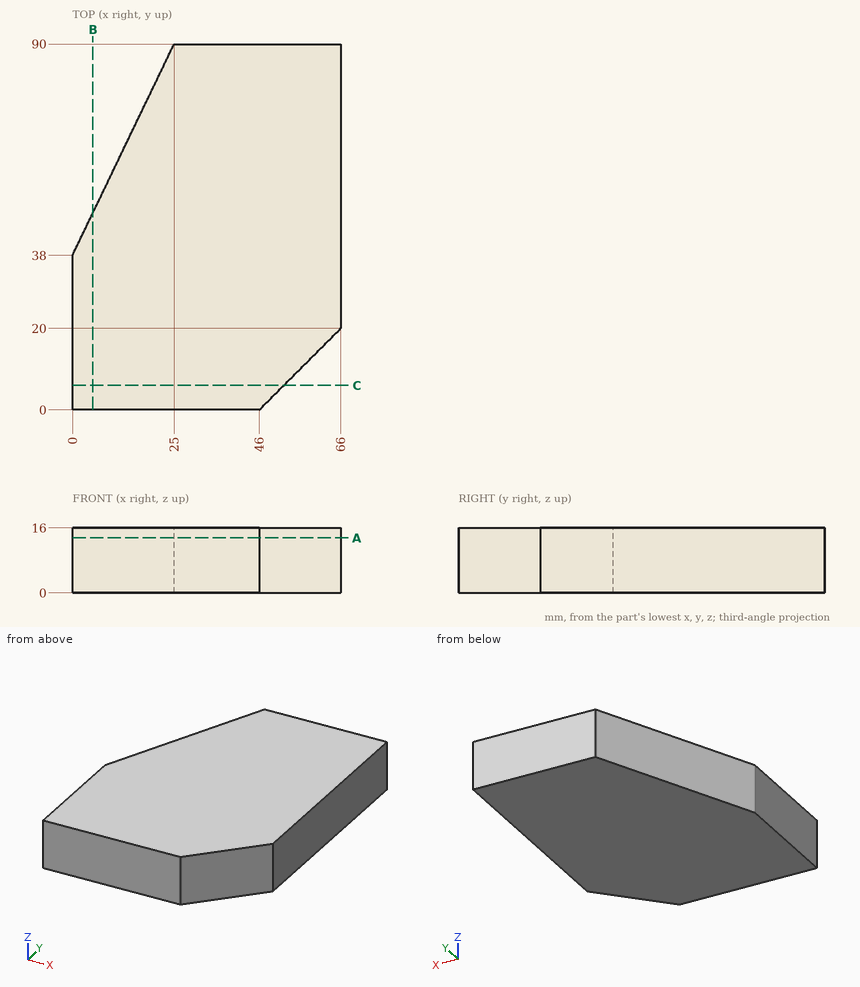
Input: dimensioned drawing with shaded views. Units: mm. Origin: part minimum x, y, z. Coordinates: 2 decimals unless noted, no trailing zeros. Loops run counter-clockwise (first coordinate to the right, second up) from the corner with the lowest first, then second, coordinate; pieces in that order, holes last. Notation, with made-up numbers: M 1.25,20.25 L 57.25,20.25 A5 cw 57.25,25.25 Z; hole C 70.5,10 d9. An arc over 180 degrees is marked long. Use a Markdown table: item, result. Add a question column.
Q1. Section query A-A, the plane z = 13.5. Return loops of the section in (x, y).
Q2. Section query C-C, the plane y = 6. Return loops of the section in (x, z), and give its area (3 significant figures).
Q3. Material intervals for L1, parallel to Y at x = 55.5, z = 1.5; L2, parallel to X at y = 7, z = 11.25; L3, parallel to Y at x = 9.5, z = 6.5, sorted ascending.
Q4. Section query B-B, the plane x = 5. Return loops of the section in (y, z).
Q5. First-contact query: pin 1 (2 mm diameter, centred on y = 50.5, z = 4.5, fed in from -X); pin 2 (5 mm diameter, centred on y = 67.5, z = 7.5, fed in from -X). Flat tips, straight axial feed; report the tip coordinate or a pass-through.
Result:
| question | item | result |
|---|---|---|
| 1 | outline | M 0,0 L 46,0 L 66,20 L 66,90 L 25,90 L 0,38 Z |
| 2 | outline | M 0,0 L 52,0 L 52,16 L 0,16 Z |
| 2 | area | 832 mm2 |
| 3 | L1 | y = 9.5 to 90 |
| 3 | L2 | x = 0 to 53 |
| 3 | L3 | y = 0 to 57.76 |
| 4 | outline | M 0,0 L 48.4,0 L 48.4,16 L 0,16 Z |
| 5 | pin 1 | stops at x = 5.53 |
| 5 | pin 2 | stops at x = 12.98 |
